Geometry check sheet. Reference: the model listing, model coordinates, mm. Round coordinates to 2 decimals unless told otherwise and drop trailing zeros. Order: outer loops, then holes, each group sorted by start corner. A loop starts at its lowest first (then second) coordinate and runs counter-clockwise, first axis right, second up.
```python
from build123d import *

# Parameters (mm, degrees)
BOSS_EXTRUDE1_DEPTH = 25
CHAMFER1_SIZE       = 15


with BuildPart() as part:
    # Sketch1 → Boss-Extrude1 (new, symmetric)
    with BuildSketch(Plane(origin=(0, 0, 0), x_dir=(0, 0, -1), z_dir=(1, 0, 0))):
        with BuildLine():
            Line((-390, 370), (390, 370))
            ThreePointArc((390, 370), (400.251262658, 345.251262658), (425, 335))
            Line((425, 335), (425, 100))
            Line((425, 100), (280, 0))
            Line((280, 0), (-280, 0))
            Line((-280, 0), (-425, 100))
            Line((-425, 100), (-425, 335))
            ThreePointArc((-425, 335), (-400.251262658, 345.251262658), (-390, 370))
        make_face()
    extrude(amount=BOSS_EXTRUDE1_DEPTH, both=True)

    # Chamfer1
    chamfer1_edges = [part.edges().sort_by_distance(p)[0] for p in [
        (-25, 370, 0),
        (25, 217.5, 425),
        (25, 217.5, -425),
        (25, 370, 0),
        (-25, 217.5, -425),
        (-25, 217.5, 425),
    ]]
    chamfer(chamfer1_edges, length=CHAMFER1_SIZE)


solid = part.part
```
(1) Sectioned sample at B-B, the plane z = -367. Record the cut outline in (x, y).
Returned:
outline: (-25, 60) - (25, 60) - (25, 355) - (10, 370) - (-10, 370) - (-25, 355) - close
(2) Depth check by flat-ended pin: P1, Ø8, axis at x = -10.5, z = 316.5, coming from the -Y side; P2, Ø12, axis at x = -15, z = 316.5, coming from the -Y side; P3, Ø10, axis at x = -14.5, y = 67, coming from the +Z side. Enter the tip coordinate at first touch or a pass-through.
Returned:
P1: stops at y = 22.41
P2: stops at y = 21.03
P3: stops at z = 384.4
(3) Material ranges on line 1 (Y direction, x = -12, z = 228); line 2 (Z direction, x = 10.5, y = 74); line 3 (Y direction, x = -14, z = -139), recorded low to high.
Returned:
line 1: y = 0 to 368
line 2: z = -387.3 to 387.3
line 3: y = 0 to 366
(4) Sectioned sample at C-C, the plane y = 52.5. Record the cut outline in (x, z) (3 decimals), and give its area (3 significant figures).
Returned:
outline: (-25, -356.125) - (25, -356.125) - (25, 356.125) - (-25, 356.125) - close
area: 35,600 mm2
(5) Sectioned sample at A-A, the plane x = -1.5. Record the cut outline in (y, z).
Returned:
outline: (0, -280) - (100, -425) - (335, -425) arc R35 cw to (370, -390) - (370, 390) arc R35 cw to (335, 425) - (100, 425) - (0, 280) - close
(6) Sectioned sample at D-D, the plane z = 318. Record the cut outline in (x, y).
Returned:
outline: (-25, 26.21) - (25, 26.21) - (25, 355) - (10, 370) - (-10, 370) - (-25, 355) - close
